Part model, mm, in its own coordinate system. Face numbers are marked on the shaded views. A direction names the side the tool comes from. Give positions to 0.01 mm unless a question says otherwise; leave off trailing zeros. Write each loop counter-clockwise with the first axis right and the second up, starting at its lowest first coordinate (ties: lowest second). Pieces come first, ordered by that corner, then holes. Notation, with made-up numbers: M -39,18.25 L 18,18.25 A28 cw 18,44.25 Z; hole C 13.25,24.5 d3. An arc over 180 degrees is marked long. Answer as CSV lines item,"result". Start each with the question number.
Item 1: Band-saw the part on A-A, the plane x = -49. List the corners of the cut face in (y, z), then the cut area to 3 significant figures.
Item 2: Pin check, flat tips, straight feed: pin 1 (1.5 mm diameter, centred on x = -22, y = 1.5, fed in from -Z); pin 2 (8 mm diameter, centred on x = -48, z = -5.5, fed in from -Y); pin 3 (2 mm diameter, centred on x = -42.5, z = 4, fed in from -Y). Stop position of each tip, or through.
Item 3: Band-saw the part on B-B, the plane y = -6.5. List the corners of the cut face in (x, z).
Item 4: Wall check: L1, parallel to X at y = 0, z = -3; L2, parallel to Y at x = -4.5, z = -0.25; L3, parallel to X at y = 0.75, z = -2.25. Give the ranges that are in metal, low to high. Write a range as from..to.
Item 5: Band-saw the part on C-C, the plane x = -10. List the corners of the cut face in (y, z), then the cut area to 3 significant figures.
Item 6: Two-plate mould, pull along Y, no slides. Class the marked faces 3, 4 and 5: +Y half, -Y half, draft (parallel to the pull), parting line (faces both ways), or undercut.
Item 7: 3-axis set-ups, long thin cutter, end or side, ignore diameter. For the marked faces 1 and 2: which of +Z, -Z, +X, -X, +Y, -Y reach the whole face in a straight line?
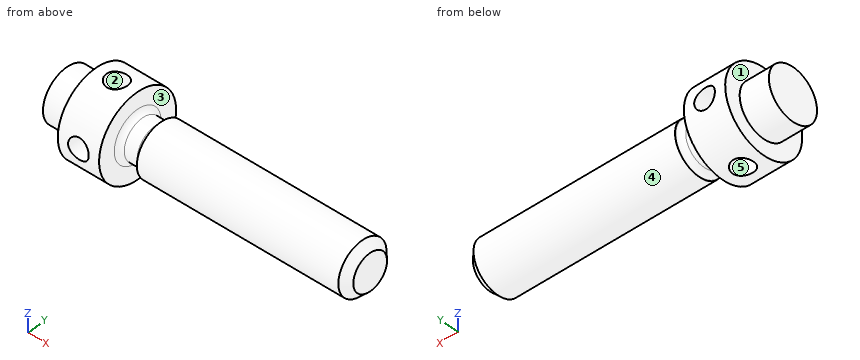
from build123d import *

# Parameters (mm, degrees)
SKETCH1_R               = 5
BOSS_EXTRUDE_DEPTH      = 40.5
CHAMFER2_SIZE           = 1.5
SKETCH2_R               = 3.85
BOSS_EXTRUDE1_DEPTH     = 4.5
SKETCH4_R               = 8
BOSS_EXTRUDE2_DEPTH     = 8
CUT_EXTRUDE1_DEPTH      = 55.194095619
CUT_EXTRUDE1_DEPTH_BACK = 55.194095619
SKETCH6_R               = 2
CUT_EXTRUDE2_DEPTH      = 55.194095747
CUT_EXTRUDE2_DEPTH_BACK = 55.194095747
SKETCH7_R               = 2
FILLET1_R               = 1
SKETCH15_W              = 10.32482264
SKETCH15_H              = 14.834361989
CUT_EXTRUDE3_DEPTH      = 21.5


with BuildPart() as part:
    # Sketch1 → Boss-Extrude (new body)
    with BuildSketch(Plane(origin=(0, 0, 0), x_dir=(0, 0, -1), z_dir=(1, 0, 0))):
        Circle(SKETCH1_R)
    extrude(amount=-BOSS_EXTRUDE_DEPTH)

    # Chamfer2
    chamfer2_edges = [part.edges().sort_by_distance(p)[0] for p in [
        (0, 0, 5),
    ]]
    chamfer(chamfer2_edges, length=CHAMFER2_SIZE)

    # Sketch2 → Boss-Extrude1 (add)
    with BuildSketch(Plane.ZY.offset(40.5)):
        with Locations(Location((0, 0, 0), (0, 0, 180))):
            Circle(SKETCH2_R)
    extrude(amount=BOSS_EXTRUDE1_DEPTH)

    # Sketch4 → Boss-Extrude2 (add)
    with BuildSketch(Plane.ZY.offset(45)):
        Circle(SKETCH4_R)
    extrude(amount=BOSS_EXTRUDE2_DEPTH)

    # Sketch6 → Cut-Extrude1 (cut, two sides: drawn at the far end of the back side and taken through both)
    with BuildSketch(Plane.XY.offset(-CUT_EXTRUDE1_DEPTH_BACK)):
        with Locations((-49, 0)):
            Circle(SKETCH6_R)
    extrude(amount=CUT_EXTRUDE1_DEPTH + CUT_EXTRUDE1_DEPTH_BACK, mode=Mode.SUBTRACT)

    # Sketch7 → Cut-Extrude2 (cut, two sides: drawn at the far end of the back side and taken through both)
    with BuildSketch(Plane(origin=(0, 0, 0), x_dir=(1, 0, 0), z_dir=(0, 1, 0)).offset(-CUT_EXTRUDE2_DEPTH_BACK)):
        with Locations(Location((-49, 0, 0), (0, 0, 270))):
            Circle(SKETCH7_R)
    extrude(amount=CUT_EXTRUDE2_DEPTH + CUT_EXTRUDE2_DEPTH_BACK, mode=Mode.SUBTRACT)

    # Sketch14 → Boss-Revolve1 (revolve)
    with BuildSketch(Plane.XY):
        with BuildLine():
            Line((-53, 0), (-53, 5))
            Line((-53, 5), (-58.660254038, 5))
            ThreePointArc((-58.660254038, 5), (-59.659258263, 2.588190451), (-60, 0))
            Line((-60, 0), (-53, 0))
        make_face()
    revolve(axis=Axis((-53, 0, 0), (-1, 0, 0)))

    # Fillet1
    fillet1_edges = [part.edges().sort_by_distance(p)[0] for p in [
        (-40.5, 0, 3.85),
        (-45, 0, 3.85),
    ]]
    fillet(fillet1_edges, radius=FILLET1_R)

    # Sketch15 → Cut-Extrude3 (cut, symmetric)
    with BuildSketch(Plane(origin=(0, 0, 0), x_dir=(1, 0, 0), z_dir=(0, 1, 0))):
        with Locations((-63.822665358, -2.417180995)):
            Rectangle(SKETCH15_W, SKETCH15_H)
    extrude(amount=CUT_EXTRUDE3_DEPTH, both=True, mode=Mode.SUBTRACT)


solid = part.part
Output:
1,outline,"M -7.75,-2 A8 ccw -2,-7.75 L -2,-2 Z; M -7.75,2 L -2,2 L -2,7.75 A8 ccw Z; M 2,-7.75 A8 ccw 7.75,-2 L 2,-2 Z; M 2,2 L 7.75,2 A8 ccw 2,7.75 Z"
1,area,"90.4 mm²"
2,pin 1,"z = -4.94"
2,pin 2,"y = -7.86"
2,pin 3,"y = -2.41"
3,outline,"M -53,-4.66 L -45,-4.66 L -45,4.66 L -53,4.66 Z; hole C -49,0 d4"
4,L1,"-58.66..-51, -47..0"
4,L2,"-4.99..4.99"
4,L3,"-58.66..-50.85, -47.15..0"
5,outline,"C 0,0 d10"
5,area,"78.5 mm²"
6,face 3,"draft"
6,face 4,"parting line"
6,face 5,"undercut"
7,face 1,"-X"
7,face 2,"+Z, -Z"
